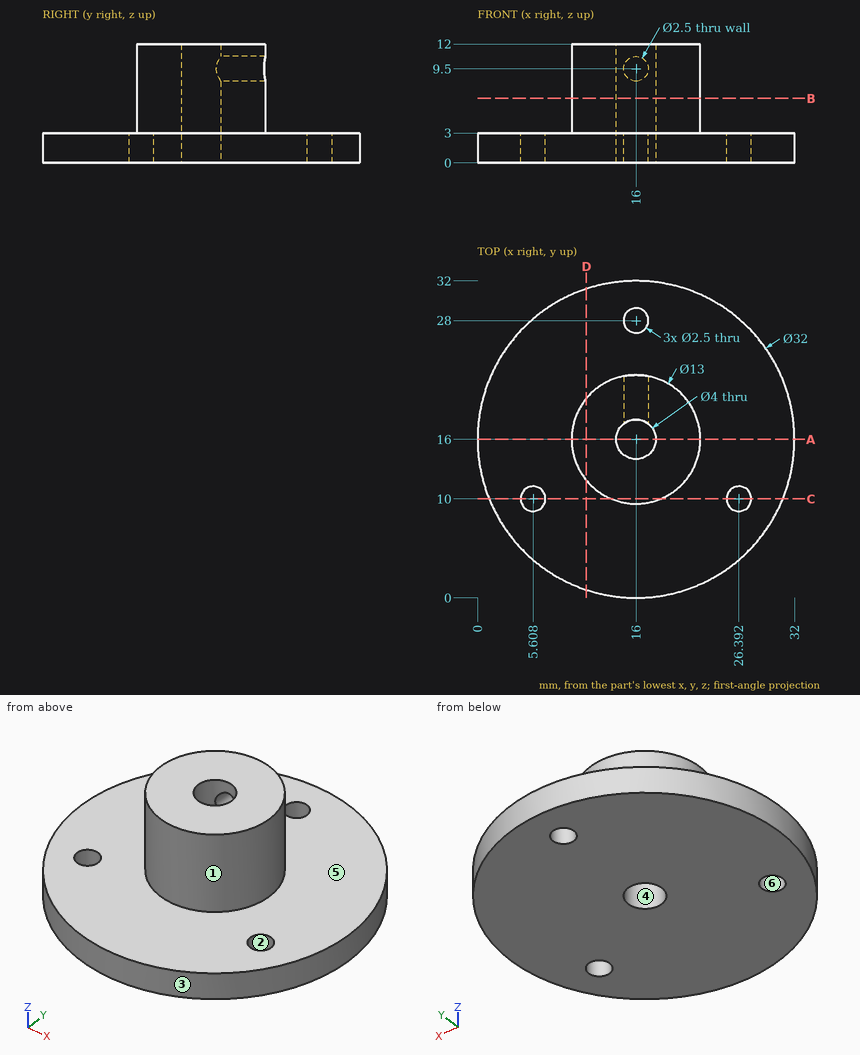
Answer from the drawing. Dimensions are ordinates in mm from the lowest x, y and z of the part. A direction names the side the tool comes from. Round coordinates to 2 decimals unless told otherwise and drop trailing zeros. Loops run counter-clockwise (first coordinate to the right, second up) from the corner with the lowest first, then second, coordinate; pieces in that order, holes last.
(1) The part is cut by section A-A, the plane y = 16. Give the vertices of the cut face in (x, z).
Computed values:
outline: (0, 0) - (14, 0) - (14, 12) - (9.5, 12) - (9.5, 3) - (0, 3) - close; (18, 0) - (32, 0) - (32, 3) - (22.5, 3) - (22.5, 12) - (18, 12) - close
(2) Find the intervals of material crossed by L1, parallel to Y at x = 16, z = 1.9; L2, parallel to Y at x = 16, z = 5; L3, parallel to Z at x = 19, y = 6, in increasing order.
Computed values:
L1: y = 0 to 14, 18 to 26.75, 29.25 to 32
L2: y = 9.5 to 14, 18 to 22.5
L3: z = 0 to 3
(3) The part is cut by section C-C, the plane y = 10. Give the vertices of the cut face in (x, z), and give its area (3 significant figures).
Computed values:
outline: (1.17, 0) - (4.36, 0) - (4.36, 3) - (1.17, 3) - close; (6.86, 0) - (25.14, 0) - (25.14, 3) - (18.5, 3) - (18.5, 12) - (13.5, 12) - (13.5, 3) - (6.86, 3) - close; (27.64, 0) - (30.83, 0) - (30.83, 3) - (27.64, 3) - close
area: 119 mm2
(4) For the marked faces 1 and 2, determine the directions among +Z, -Z, +X, -X, +Y, -Y from which every point of the face is accessible in a straight line to the end or side of a thin tool.
Computed values:
face 1: +Z
face 2: +Z, -Z
(5) The mould has two halves that part along Y. Classify the marked faces 3, 4, 5 and 6: pulls with the +Y half, pulls with the -Y half, needs draft (parallel to the pull), parting line crosses it, or undercut.
Computed values:
face 3: parting line crosses it
face 4: undercut
face 5: needs draft
face 6: undercut
(6) Each of these flat-tipped pins is pushed along its axis until it touches: P1, Ø4, axis at y = 9.5, z = 10, coming from the +X side; P2, Ø5, axis at x = 24.5, z = 10.5, coming from the +Y side; P3, Ø3.5, axis at x = 16, y = 16, coming from the -Z side; P4, Ø2, axis at x = 16, z = 9.5, coming from the +Y side. Where does it stop, or does it pass through?
Computed values:
P1: stops at x = 20.69
P2: stops at y = 18.5
P3: passes through
P4: stops at y = 14.27
(7) The part is cut by section B-B, the plane z = 6.5. Give the vertices of the cut face in (x, y).
Computed values:
outline: circle Ø13 at (16, 16); hole circle Ø4 at (16, 16)
(8) The part is cut by section D-D, the plane x = 11. Give the vertices of the cut face in (y, z), and give its area (3 significant figures).
Computed values:
outline: (0.8, 0) - (31.2, 0) - (31.2, 3) - (20.15, 3) - (20.15, 12) - (11.85, 12) - (11.85, 3) - (0.8, 3) - close
area: 166 mm2
